Work out the finished part from the listing and answer in its coordinate system (mm). A direction names the side the tool comes from. Round coordinates to 2 decimals unless told otherwise and drop trailing zeros. Order: outer loops, then holes, each group sorted by start corner. A loop starts at its lowest first (then second) coordinate and runs counter-clockwise, first axis right, second up. Notation, with made-up numbers: (26.25, -6) -> (85.25, -6) arc R19 ccw to (85.25, 6) -> close; hole circle Ø11 at (-25.75, 54.5). An arc over 180 degrees is marked (long way). Use a Markdown table: item, result. Add a question column.
Item 1: A cutting plane is placed at A-A, the plane y = 43.5. Determine the outline of the cut face in (x, z).
Item 2: A cutting plane is placed at C-C, the plane y = -8.5. Determine the outline of the cut face in (x, z), plus the area to 3 significant figures.
Item 3: Find the intervals of material crossed by L1, parallel to X at y = -5.5, z = -0.75; L2, parallel to X at y = 39.5, z = -0.5; L3, parallel to X at y = -36.5, z = 1.5, in increasing order. Write a range as [from, to].
Item 4: A cutting plane is placed at B-B, the plane z = -2.25. Determine the outline of the cut face in (x, y).
Item 5: For a pull along X with two mould halves and no side action, classify faces 1 (the flat face through (-9, -64, 4)), 2 (the flat face through (-13.993, -62, -2)), 3 (the cylindrical face through (-9.1, -70.98, -2.08)) as +X half, -X half, draft (parallel to the pull), parting line (faces both ways), or undercut.
Item 6: A cutting plane is placed at D-D, the plane x = 44.5. Determine the outline of the cut face in (y, z), plus the area to 3 significant figures.
Item 7: Flat-ended cylindrical pins translate along their axes: P1, Ø1, axis at x = -1, y = -25.5, coming from the -Z side; P2, Ø3, axis at x = -48, y = -5.5, coming from the +Z side; P3, Ø5, axis at x = 9, z = 2.5, coming from the -Y side. Find the tip coordinate at first contact, or state that the pin passes through.
Item 8: A tool of negligible diameter and unlimited length cuts with its end or side. For faces 4 (the flat face through (98.007, 43, -2)), 5 (the flat face through (-3.993, -62, -2)), 6 (the flat face through (-48, -0.983, -2)), from which of +Z, -Z, +X, -X, +Y, -Y can it reach the whole face along a straight path? Write none if from no direction.
from build123d import *

# Parameters (mm, degrees)
SKETCH1_W           = 182
SKETCH1_H           = 97
BOSS_EXTRUDE1_DEPTH = 6
BOSS_EXTRUDE2_DEPTH = 12


with BuildPart() as part:
    # Sketch1 → Boss-Extrude1 (new body)
    with BuildSketch(Plane.XY):
        with Locations((47.006685832, -9.482901158)):
            Rectangle(SKETCH1_W, SKETCH1_H)
    extrude(amount=BOSS_EXTRUDE1_DEPTH)

    # Sketch2 → Boss-Extrude2 (add)
    with BuildSketch(Plane.XY.offset(-8)):
        with BuildLine():
            Line((108.006685832, -65.982901158), (108.006685832, -57.982901158))
            Line((108.006685832, -57.982901158), (98.006685832, -57.982901158))
            Line((98.006685832, -57.982901158), (98.006685832, -65.982901158))
            ThreePointArc((98.006685832, -65.982901158), (103.006685832, -70.982901158), (108.006685832, -65.982901158))
        make_face()
        with BuildLine():
            Line((138.006685832, -0.982901158), (138.006685832, -10.982901158))
            Line((138.006685832, -10.982901158), (146.006685832, -10.982901158))
            ThreePointArc((146.006685832, -10.982901158), (151.006685832, -5.982901158), (146.006685832, -0.982901158))
            Line((146.006685832, -0.982901158), (138.006685832, -0.982901158))
        make_face()
        with BuildLine():
            Line((108.006685832, 39.017098842), (108.006685832, 47.017098842))
            ThreePointArc((108.006685832, 47.017098842), (103.006685832, 52.017098842), (98.006685832, 47.017098842))
            Line((98.006685832, 47.017098842), (98.006685832, 39.017098842))
            Line((98.006685832, 39.017098842), (108.006685832, 39.017098842))
        make_face()
        with BuildLine():
            Line((-13.993314168, 47.017098842), (-13.993314168, 39.017098842))
            Line((-13.993314168, 39.017098842), (-3.993314168, 39.017098842))
            Line((-3.993314168, 39.017098842), (-3.993314168, 47.017098842))
            ThreePointArc((-3.993314168, 47.017098842), (-8.993314168, 52.017098842), (-13.993314168, 47.017098842))
        make_face()
        with BuildLine():
            Line((-43.993314168, -10.982901158), (-43.993314168, -0.982901158))
            Line((-43.993314168, -0.982901158), (-51.993314168, -0.982901158))
            ThreePointArc((-51.993314168, -0.982901158), (-56.993314168, -5.982901158), (-51.993314168, -10.982901158))
            Line((-51.993314168, -10.982901158), (-43.993314168, -10.982901158))
        make_face()
        with BuildLine():
            Line((-13.993314168, -57.982901158), (-13.993314168, -65.982901158))
            ThreePointArc((-13.993314168, -65.982901158), (-8.993314168, -70.982901158), (-3.993314168, -65.982901158))
            Line((-3.993314168, -65.982901158), (-3.993314168, -57.982901158))
            Line((-3.993314168, -57.982901158), (-13.993314168, -57.982901158))
        make_face()
    extrude(amount=BOSS_EXTRUDE2_DEPTH)


solid = part.part
Reported:
| question | item | result |
|---|---|---|
| 1 | outline | (-13.99, -8) -> (-3.99, -8) -> (-3.99, 4) -> (-13.99, 4) -> close; (98.01, -8) -> (108.01, -8) -> (108.01, 4) -> (98.01, 4) -> close |
| 2 | outline | (-56.31, -8) -> (-43.99, -8) -> (-43.99, 0) -> (138.01, 0) -> (138.01, -8) -> (150.33, -8) -> (150.33, 4) -> (138.01, 4) -> (138.01, 6) -> (-43.99, 6) -> (-43.99, 4) -> (-56.31, 4) -> close |
| 2 | area | 1,390 mm² |
| 3 | L1 | [-56.97, -43.99], [138.01, 150.98] |
| 3 | L2 | [-13.99, -3.99], [98.01, 108.01] |
| 3 | L3 | [-43.99, 138.01] |
| 4 | outline | (-51.99, -10.98) -> (-43.99, -10.98) -> (-43.99, -0.98) -> (-51.99, -0.98) arc R5 ccw to start; (-13.99, -65.98) arc R5 ccw to (-3.99, -65.98) -> (-3.99, -57.98) -> (-13.99, -57.98) -> close; (-13.99, 39.02) -> (-3.99, 39.02) -> (-3.99, 47.02) arc R5 ccw to (-13.99, 47.02) -> close; (98.01, -65.98) arc R5 ccw to (108.01, -65.98) -> (108.01, -57.98) -> (98.01, -57.98) -> close; (98.01, 39.02) -> (108.01, 39.02) -> (108.01, 47.02) arc R5 ccw to (98.01, 47.02) -> close; (138.01, -10.98) -> (146.01, -10.98) arc R5 ccw to (146.01, -0.98) -> (138.01, -0.98) -> close |
| 5 | face 1 | draft |
| 5 | face 2 | -X half |
| 5 | face 3 | undercut |
| 6 | outline | (-57.98, 0) -> (39.02, 0) -> (39.02, 6) -> (-57.98, 6) -> close |
| 6 | area | 582 mm² |
| 7 | P1 | z = 0 |
| 7 | P2 | z = 4 |
| 7 | P3 | y = -57.98 |
| 8 | face 4 | +Z, -Z, +Y |
| 8 | face 5 | +Z, -Z, -Y |
| 8 | face 6 | +Z, -Z, -X, +Y |
